```python
from build123d import *

# Parameters (mm, degrees)
CHAMFER_1_SIZE = 1


with BuildPart() as part:
    # 草图1 → 旋转1 (revolve)
    with BuildSketch(Plane.XY, mode=Mode.PRIVATE) as revolve_1_sk:
        Polygon((349.087142185, 76.281973739), (349.087142185, 69.281973739), (348.087142185, 69.281973739), (348.087142185, 66.281973739), (349.737142185, 66.281973739), (349.737142185, 40.081973739), (355.587142185, 40.081973739), (355.587142185, 30.081973739), (343.087142185, 30.081973739), (343.087142185, 76.281973739), align=None)
    revolve(revolve_1_sk.sketch.rotate(Axis((343.087142185, 30.081973739, 0), (0, 1, 0)), 90), axis=Axis((343.087142185, 30.081973739, 0), (0, 1, 0)))

    # 倒角1
    chamfer_1_edges = [part.edges().sort_by_distance(p)[0] for p in [
        (343.087142185, 66.281973739, 6.65),
        (343.087142185, 30.081973739, 12.5),
        (343.087142185, 40.081973739, 12.5),
    ]]
    chamfer(chamfer_1_edges, length=CHAMFER_1_SIZE)


solid = part.part
```
For this review, take the finished solid that the model builds, in its own axes (mm). A direction names the side the tool comes from. Round coordinates to 2 decimals unless told otherwise and drop trailing zeros. Loops run counter-clockwise (first coordinate to the right, second up) from the corner with the lowest first, then second, coordinate; pieces in that order, holes last.
(1) Wall thickness on line 1 along Y through (x, z) = (343.5, 9.75); line 2 along Y through (x, z) = (339.5, -3.75); line 3 along X through (y, z) = (53, -1): over which ranges is each line inside the solid? List them lowest first.
Returned:
line 1: y = 30.08 to 40.08
line 2: y = 30.08 to 66.28, 69.28 to 76.28
line 3: x = 336.51 to 349.66
(2) Clearance check with flat-ended pins moving along their axes: P1, Ø2, axis at y = 37.5, z = -9.5, coming from the -X side; P2, Ø8, axis at y = 36.5, z = 4, coming from the -X side; P3, Ø10, axis at x = 340.5, y = 59, coming from the +Z side; P4, Ø8, axis at x = 339.5, y = 64.5, coming from the -Z side. State where each tip first meets the part, or that it passes through.
Returned:
P1: stops at x = 333.92
P2: stops at x = 330.59
P3: stops at z = 6.65
P4: stops at z = -6.65
(3) Tool access review of faces 5 (the cylindrical face through (338.03, 72.73, -3.23)), 6 (the cylindrical face through (330.694, 35.026, 1.627)), 7 (the flat face through (338, 69.282, 1)): name each direction out of +Z, -Z, +X, -X, +Y, -Y from which nothing blocks a thin tool from reaching the whole face with its end or side.
Returned:
face 5: +Y
face 6: +Y, -Y
face 7: none
(4) We need section B-B (y = 34.5). Give the boundary of the cut face in (x, z).
Returned:
outline: circle Ø25 at (343.09, 0)
(5) We need section C-C (y = 54). Give the boundary of the cut face in (x, z), plus the area to 3 significant figures.
Returned:
outline: circle Ø13.3 at (343.09, 0)
area: 139 mm2
(6) We need section A-A (z = 0). Give the boundary of the cut face in (x, y), plus the area to 3 significant figures.
Returned:
outline: (330.59, 31.08) - (331.59, 30.08) - (354.59, 30.08) - (355.59, 31.08) - (355.59, 39.08) - (354.59, 40.08) - (349.74, 40.08) - (349.74, 65.28) - (348.74, 66.28) - (348.09, 66.28) - (348.09, 69.28) - (349.09, 69.28) - (349.09, 76.28) - (337.09, 76.28) - (337.09, 69.28) - (338.09, 69.28) - (338.09, 66.28) - (337.44, 66.28) - (336.44, 65.28) - (336.44, 40.08) - (331.59, 40.08) - (330.59, 39.08) - close
area: 709 mm2
(7) Mouldability with a two-part tool opening along Y and no side actions: class faces 1 (the flat face through (348, 40.082, 5)), 2 (the cylindrical face through (347.52, 67.76, -2.31)), 3 (the cylindrical face through (349.58, 52.51, 1.44)), 4 (the flat face through (343, 30.082, 0)) as released by +Y, released by -Y, zero draft, split by the parting line, or undercut.
Returned:
face 1: released by +Y
face 2: undercut
face 3: zero draft
face 4: released by -Y
